Build history of the part. All positions in model axes, mm. A direction names the side the tool comes from. Give positions to 0.01 mm unless a question says otherwise; leave off trailing zeros. Write each loop counter-clockwise with the first axis right and the second up, starting at its lowest first coordinate (ties: lowest second). Pieces come first, ordered by that corner, then holes. Notation, with made-up numbers: (24.25, 12.25) -> (79.25, 12.25) arc R25 cw to (79.25, 32.25) -> close; hole circle Ø7 at (-36, 49). An arc over 180 degrees is marked (long way). Put each result on its own line as item: value. Start each with the question number.
Item 1: Slice it at B-B, the plane z = -4. List the corners of the cut face in (x, y).
Item 2: Flat gauge pins, fed straight in: pin 1 Ø16 at (y, z) = (82, -11) entering from -X; pin 2 Ø5 at (x, y) = (98.5, 82.5) entering from -Z; pin 3 Ø6 at (y, z) = (54.5, -8) entering from +X. Where does each tip first touch, or does it go through?
Item 3: Drill centre lines: line 1 along X through (y, z) = (64.5, -11); line 2 along Z through (x, y) = (430, 93). Where is each one in solid material? Low to high.
Item 4: Slice it at A-A, the plane y = 52. List the corners of the cut face in (x, z), plus the area to 3 significant figures.
Item 5: Slice it at C-C, the plane x = 58. List the corners of the cut face in (y, z).
Item 6: Tool access for faces 1 (the flat face through (228, 74, 40)), 2 (the flat face through (335, 74, -10)), 3 (the flat face through (115, 74, -10)): list every direction of +Z, -Z, +X, -X, +Y, -Y with a clear straight run to the whole face (end or side of a thin tool).
```python
from build123d import *

# Parameters (mm, degrees)
BOSS_EXTRUDE1_DEPTH = 150


with BuildPart() as part:
    # Sketch1 → Boss-Extrude1 (new body)
    with BuildSketch(Plane(origin=(0, 0, 0), x_dir=(1, 0, 0), z_dir=(0, 1, 0))):
        Polygon((115, 0), (115, 20), (335, 20), (335, 0), (450, 0), (450, -40), (0, -40), (0, 0), align=None)
    extrude(amount=BOSS_EXTRUDE1_DEPTH)


solid = part.part
```
Values follow:
1. outline: (115, 0) -> (335, 0) -> (335, 150) -> (115, 150) -> close
2. pin 1: x = 115
2. pin 2: z = 0
2. pin 3: x = 335
3. line 1: 115 to 335
3. line 2: 0 to 40
4. outline: (0, 0) -> (115, 0) -> (115, -20) -> (335, -20) -> (335, 0) -> (450, 0) -> (450, 40) -> (0, 40) -> close
4. area: 22,400 mm2
5. outline: (0, 0) -> (150, 0) -> (150, 40) -> (0, 40) -> close
6. face 1: +Z, +X, -X, +Y, -Y
6. face 2: -Z, +X, +Y, -Y
6. face 3: -Z, -X, +Y, -Y
